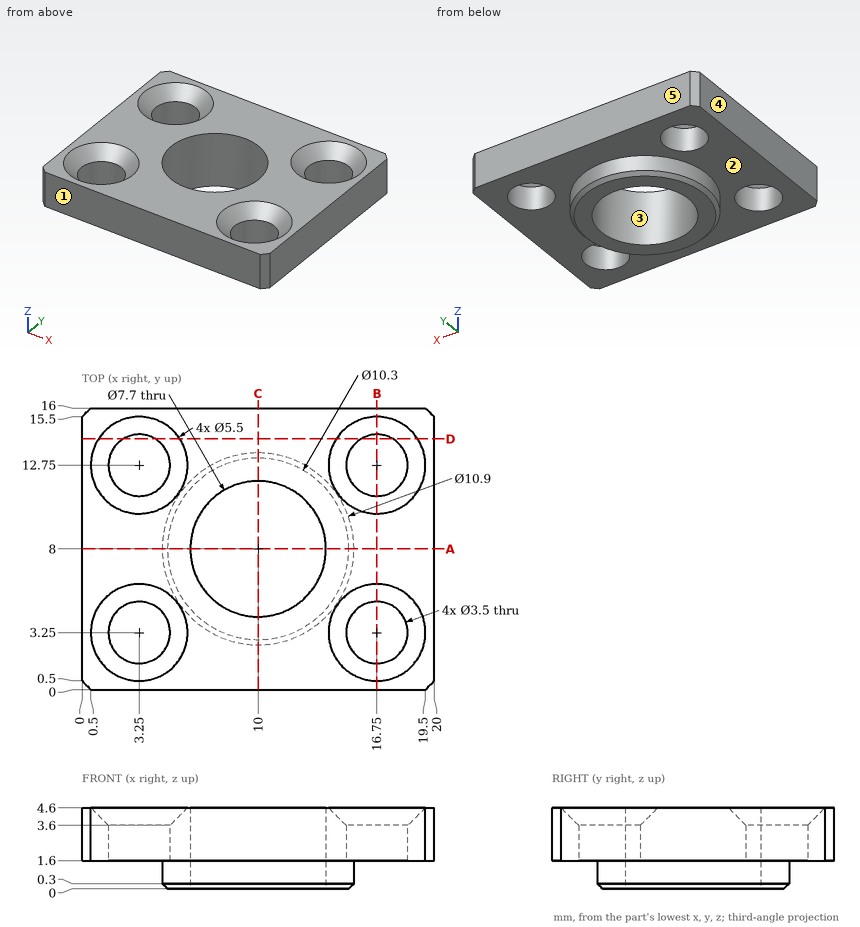
Study the drawing (mm; zero at the part's minimum x, y, z) and answer. A direction names the side the tool comes from. Coordinates: 2 decimals unless noted, no trailing zeros. Loops run counter-clockwise (first coordinate to the right, second up) from the corner with the lowest first, then second, coordinate; pieces in that order, holes last. Notation, with made-up numbers: (-2.75, 29.25) -> (40.25, 29.25) arc R19 ccw to (40.25, 57.25) -> close; hole circle Ø2 at (61.25, 73). An arc over 180 degrees is marked (long way). Write each question's results on one line, items separated by ' | '. Start each with the question number.
1) The mould has two halves that part along X. Classify the marked faces 3, 4 and 5: pulls with the +X half, pulls with the -X half, needs draft (parallel to the pull), parting line crosses it, or undercut.
2) Find section D-D on y = 14.25. Count the separate pieces of the cut face and the enclosed holes in it, then the cut area to 3 significant figures.
3) Find section C-C on x = 10. Determine the outline of the cut face in (y, z).
4) Flat-ended cylindrical pins translate along their axes: P1, Ø2, axis at x = 3.25, y = 12.75, coming from the -Z side; P2, Ø2, axis at x = 12.5, z = 1.5, coming from the +Y side; P3, Ø5.5, axis at x = 16.75, y = 3.25, coming from the -Z side. Find the tip coordinate at first contact, or state that the pin passes through.
5) Consider line 1 along Y through (x, z) = (16.75, 2.55); line 2 along X through (y, z) = (3, 2.2); line 3 along Y through (x, z) = (10, 1.4). Determine where each line is inside the solid, lowest interval first.
6) Find section A-A on y = 8. Determine the outline of the cut face in (x, z), then the cut area to 3 significant figures.
7) For the marked faces 1 and 2, determine the directions among +Z, -Z, +X, -X, +Y, -Y from which every point of the face is accessible in a straight line to the end or side of a thin tool.
8) Find section B-B on x = 16.75. Determine the outline of the cut face in (y, z).
Response values:
1) face 3: undercut | face 4: pulls with the -X half | face 5: needs draft
2) separate pieces: 3 | enclosed holes: 0 | area: 46.2 mm^2
3) outline: (0, 1.6) -> (2.55, 1.6) -> (2.55, 0.3) -> (2.85, 0) -> (4.15, 0) -> (4.15, 4.6) -> (0, 4.6) -> close; (11.85, 0) -> (13.15, 0) -> (13.45, 0.3) -> (13.45, 1.6) -> (16, 1.6) -> (16, 4.6) -> (11.85, 4.6) -> close
4) P1: passes through | P2: stops at y = 16 | P3: stops at z = 1.6
5) line 1: y = 0 to 1.5, 5 to 11, 14.5 to 16 | line 2: x = 0 to 1.52, 4.98 to 15.02, 18.48 to 20 | line 3: y = 2.55 to 4.15, 11.85 to 13.45
6) outline: (0, 1.6) -> (4.55, 1.6) -> (4.55, 0.3) -> (4.85, 0) -> (6.15, 0) -> (6.15, 4.6) -> (0, 4.6) -> close; (13.85, 0) -> (15.15, 0) -> (15.45, 0.3) -> (15.45, 1.6) -> (20, 1.6) -> (20, 4.6) -> (13.85, 4.6) -> close | area: 41.9 mm^2
7) face 1: +Z, -Z, +X, -X, -Y | face 2: -Z
8) outline: (0, 1.6) -> (1.5, 1.6) -> (1.5, 3.6) -> (0.5, 4.6) -> (0, 4.6) -> close; (5, 1.6) -> (11, 1.6) -> (11, 3.6) -> (10, 4.6) -> (6, 4.6) -> (5, 3.6) -> close; (14.5, 1.6) -> (16, 1.6) -> (16, 4.6) -> (15.5, 4.6) -> (14.5, 3.6) -> close
